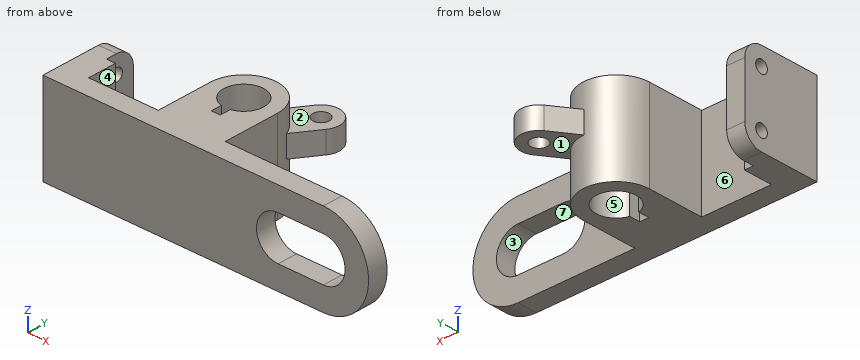
from build123d import *

# Parameters (mm, degrees)
SLOTTED_BASE_PLATE_DEPTH = 11
UPRIGHT_HUB_BODY_DEPTH   = 50
CROSS_START              = 12
CROSS_BOSS_SKETCH_R      = 4.5
CROSS_BOSS_DEPTH         = 12
UPRIGHT_FILLET_R10_R     = 10
CROSS_HOLE_SKETCH_R      = 3.5
CROSS_HOLE_CUT_DEPTH     = 12


with BuildPart() as part:
    # Base Plate Sketch → Slotted Base Plate (new body)
    with BuildSketch(Plane(origin=(0, 0, 0), x_dir=(1, 0, 0), z_dir=(0, 1, 0))):
        with BuildLine():
            Line((0, 25), (-155, 25))
            Line((-155, 25), (-155, -25))
            Line((-155, -25), (0, -25))
            ThreePointArc((0, -25), (25, 0), (0, 25))
        make_face()
        with BuildLine():
            Line((0, -12), (-25, -12))
            ThreePointArc((-25, -12), (-37, 0), (-25, 12))
            Line((-25, 12), (0, 12))
            ThreePointArc((0, 12), (12, 0), (0, -12))
        make_face(mode=Mode.SUBTRACT)
    extrude(amount=SLOTTED_BASE_PLATE_DEPTH)

    # Upright Profile Sketch → Upright Hub Body (add)
    # profile 1 of 2: a face of its own
    with BuildSketch(Plane.XY.offset(25)):
        Polygon((-155, 0), (-155, 43), (-145, 43), (-145, 27), (-140, 27), (-140, 11), align=None)
    # profile 2 of 2: a face of its own
    with BuildSketch(Plane.XY.offset(25)):
        with BuildLine():
            Line((-101.5, 42), (-101.5, 11))
            Line((-101.5, 11), (-64.5, 11))
            Line((-64.5, 11), (-64.5, 42))
            ThreePointArc((-64.5, 42), (-83, 60.5), (-101.5, 42))
        make_face()
        with BuildLine():
            Line((-85.5, 25.287857357), (-80.5, 25.287857357))
            Line((-80.5, 25.287857357), (-80.5, 31.287857357))
            ThreePointArc((-80.5, 31.287857357), (-83, 53), (-85.5, 31.287857357))
            Line((-85.5, 31.287857357), (-85.5, 25.287857357))
        make_face(mode=Mode.SUBTRACT)
    extrude(amount=-UPRIGHT_HUB_BODY_DEPTH)

    # Cross Boss Sketch → Cross Boss (add)
    with BuildSketch(Plane.XY.offset(CROSS_START)):
        with BuildLine():
            Line((-65.881116557, 49.013831311), (-56.454033594, 62.477101054))
            ThreePointArc((-56.454033594, 62.477101054), (-58.909789673, 76.40438586), (-72.83707448, 73.948629781))
            Line((-72.83707448, 73.948629781), (-82.264157443, 60.485360038))
            ThreePointArc((-82.264157443, 60.485360038), (-72.388835928, 57.154312819), (-65.881116557, 49.013831311))
        make_face()
        with Locations((-64.645554037, 68.212865417)):
            Circle(CROSS_BOSS_SKETCH_R, mode=Mode.SUBTRACT)
    extrude(amount=-CROSS_BOSS_DEPTH)

    # Upright Fillet R10
    upright_fillet_r10_edges = [part.edges().sort_by_distance(p)[0] for p in [
        (-150, 43, 25),
        (-150, 43, -25),
    ]]
    fillet(upright_fillet_r10_edges, radius=UPRIGHT_FILLET_R10_R)

    # Cross Hole Sketch → Cross Hole Cut (cut)
    with BuildSketch(Plane.ZY.offset(155)):
        with Locations((15, 33)):
            Circle(CROSS_HOLE_SKETCH_R)
        with Locations((-15, 33)):
            Circle(CROSS_HOLE_SKETCH_R)
    extrude(amount=-CROSS_HOLE_CUT_DEPTH, mode=Mode.SUBTRACT)


solid = part.part
CAD build for the part. Positions are in the model's coordinates, mm. Face numbers are marked on the shaded views. A direction names the side the tool comes from. Round coordinates to 2 decimals unless told otherwise and drop trailing zeros. Write each loop counter-clockwise with the first axis right and the second up, starting at its lowest first coordinate (ties: lowest second). Pieces come first, ordered by that corner, then holes.
(1) Slice it at A-A, the plane x = -7. Write the cut outline in (y, z).
(2) 3-axis set-ups, long thin cutter, end or side, ignore diameter. For the marked faces 1, 2, 3 and 4: which of +Z, -Z, +X, -X, +Y, -Y reach the whole face in a straight line?
(3) Probe line 1 along X through (y, z) = (42, -8); line 2 along X through (y, z) = (31, -0.5); line 3 along Y through (x, z) = (-83, -0.5). List the from-to ranges inside material, lowest first.
(4) Drop flat-ended pins along their axis: P1, Ø1.5, axis at x = -141.5, z = 9.5, coming from the +Y side; P2, Ø15, axis at x = -29, z = -1.5, coming from the +Y side; P3, Ø5, axis at y = 35.5, z = 4, coming from the +X side; P4, Ø5, axis at y = 61.5, z = -7.5, coming from the -X side. Give the stop position or say it passes through.
(5) Slice it at D-D, the plane z = 7. Write the cut outline in (x, y), and give its area (3 significant figures).
(6) Slice it at B-B, the plane z = -8. Write the cut outline in (x, y).
(7) Mould opens along Y. For the marked faces 5, 6 and 7 say: pulls with the +Y half, pulls with the -Y half, needs draft (parallel to the pull), parting line crosses it, or undercut.
(8) Slice it at C-C, the plane y = 8.5. Write the cut outline in (x, z).
From the geometry:
1. outline: (0, -25) - (11, -25) - (11, -12) - (0, -12) - close; (0, 12) - (11, 12) - (11, 25) - (0, 25) - close
2. face 1: -Z, +X, +Y
2. face 2: +Z, +X, +Y
2. face 3: +Y, -Y
2. face 4: +Z, -Z, +Y
3. line 1: x = -155 to -145, -101.5 to -94, -72 to -64.5
3. line 2: x = -155 to -145, -101.5 to -85.5, -80.5 to -64.5
3. line 3: y = 0 to 25.29, 53 to 60.5
4. P1: stops at y = 27
4. P2: passes through
4. P3: stops at x = -64.5
4. P4: stops at x = -90.3
5. outline: (-155, 0) - (-34.75, 0) - (-34.75, 11) - (-64.5, 11) - (-64.5, 42) arc R18.5 ccw to (-65.88, 49.01) - (-56.45, 62.48) arc R10 ccw to (-72.84, 73.95) - (-82.26, 60.49) arc R18.5 ccw to (-101.5, 42) - (-101.5, 11) - (-140, 11) - (-140, 27) - (-145, 27) - (-145, 43) - (-155, 43) - close; (9.75, 0) - (24, 0) - (24, 11) - (9.75, 11) - close; hole (-85.5, 25.29) - (-80.5, 25.29) - (-80.5, 31.29) arc R11 ccw (long way) to (-85.5, 31.29) - close; hole circle Ø9 at (-64.65, 68.21)
5. area: 3,540 mm2
6. outline: (-155, 0) - (-33.94, 0) - (-33.94, 11) - (-64.5, 11) - (-64.5, 42) arc R18.5 ccw to (-101.5, 42) - (-101.5, 11) - (-140, 11) - (-140, 27) - (-145, 27) - (-145, 43) - (-155, 43) - close; (8.94, 0) - (23.69, 0) - (23.69, 11) - (8.94, 11) - close; hole (-85.5, 25.29) - (-80.5, 25.29) - (-80.5, 31.29) arc R11 ccw (long way) to (-85.5, 31.29) - close
7. face 5: undercut
7. face 6: pulls with the +Y half
7. face 7: needs draft
8. outline: (-155, -25) - (0, -25) arc R25 ccw to (0, 25) - (-155, 25) - close; hole (-25, -12) - (0, -12) arc R12 ccw to (0, 12) - (-25, 12) arc R12 ccw to start
